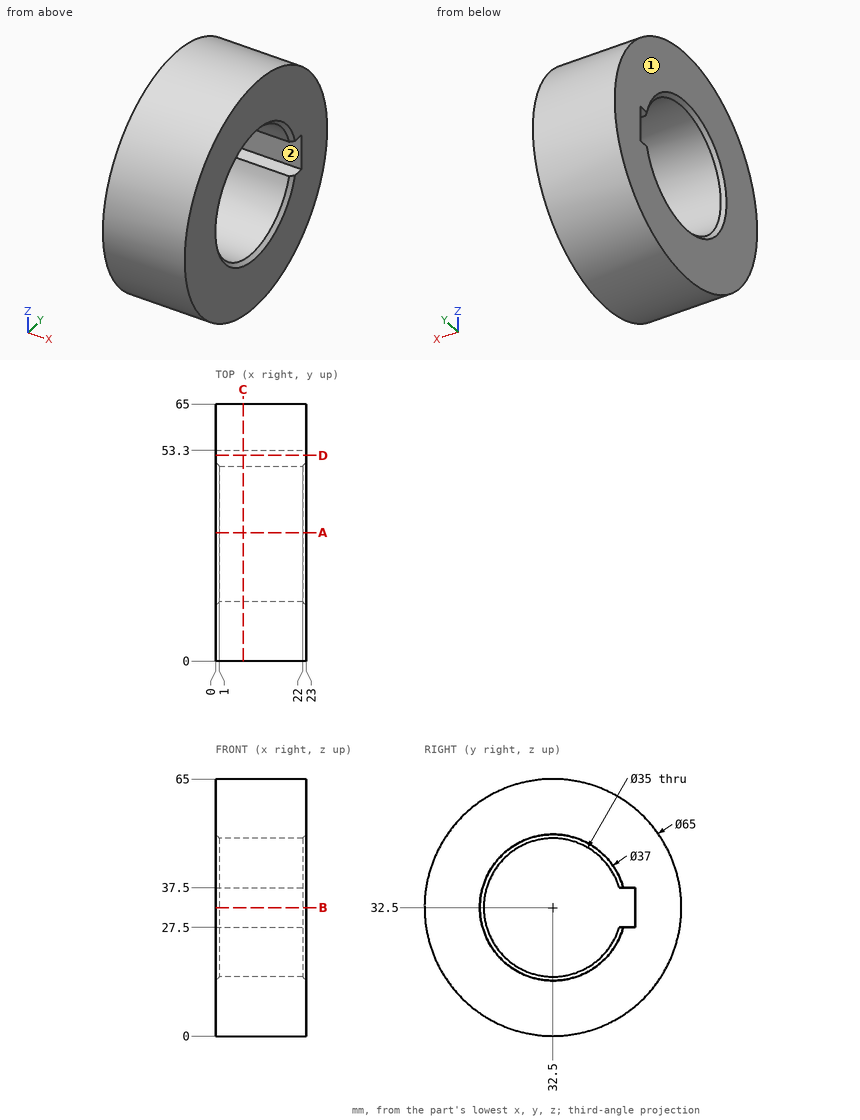
For this review, use the dimensioned drawing (mm, ordinates from the lowest corner) and the shaded views. A direction names the side the tool comes from. Round coordinates to 2 decimals unless told otherwise and drop trailing zeros. Order: outer loops, then holes, each group sorted by start corner. A loop starts at its lowest first (then second) coordinate and runs counter-clockwise, first axis right, second up. Notation, with made-up numbers: M 72.5,36.25 L 105.5,36.25 A8 cw 105.5,50.25 Z; hole C 74.5,68.5 d5. An arc over 180 degrees is marked long. Use a Markdown table: item, result.
1) Consider section D-D (y = 52). Write out the cut boundary in (x, z).
Report:
| item | result |
|---|---|
| outline | M 0,6.5 L 23,6.5 L 23,27.5 L 0,27.5 Z; M 0,37.5 L 23,37.5 L 23,58.5 L 0,58.5 Z |
2) Tool access review of the marked faces 1 and 2: name each direction out of +Z, -Z, +X, -X, +Y, -Y from which nothing blocks a thin tool from reaching the whole face with its end or side.
Report:
| item | result |
|---|---|
| face 1 | +Z, -Z, -X, +Y, -Y |
| face 2 | +X, -X |
3) Consider section C-C (x = 7). Write out the cut boundary in (y, z), then the cut area to 3 significant figures.
Report:
| item | result |
|---|---|
| outline | C 32.5,32.5 d65; hole M 49.27,27.5 L 53.3,27.5 L 53.3,37.5 L 49.27,37.5 A17.5 ccw long Z |
| area | 2,320 mm^2 |
4) Consider section B-B (z = 32.5). Write out the cut boundary in (x, y), then the cut area to 3 significant figures.
Report:
| item | result |
|---|---|
| outline | M 0,0 L 23,0 L 23,14 L 22,15 L 1,15 L 0,14 Z; M 0,53.3 L 23,53.3 L 23,65 L 0,65 Z |
| area | 613 mm^2 |
5) Consider section A-A (y = 32.5). Write out the cut boundary in (x, z).
Report:
| item | result |
|---|---|
| outline | M 0,0 L 23,0 L 23,14 L 22,15 L 1,15 L 0,14 Z; M 0,51 L 1,50 L 22,50 L 23,51 L 23,65 L 0,65 Z |
6) Wall thickness on line 1 along Y through (x, z) = (7, 32.5); line 2 along Z through (x, y) = (2.75, 50); line 3 along Y through (x, z) = (7.5, 21): over which ranges is each line inside the solid? List them lowest first. Write a range as [from, to].
Report:
| item | result |
|---|---|
| line 1 | [0, 15], [53.3, 65] |
| line 2 | [5.11, 27.5], [37.5, 59.89] |
| line 3 | [2.1, 19.31], [45.69, 62.9] |
7) Insertion check: pin 1 (6 mm diameter, centred on x = 19.5, z = 37.5, fed in from +Y); pin 2 (1.2 mm diameter, centred on x = 8, y = 52, fed in from +Z); pin 3 (1.2 mm diameter, centred on x = 9.5, y = 51, fed in from -Z); pin 4 (5 mm diameter, centred on y = 37, z = 17, fed in from +X). Each pin has a flat end and moves straight along its axis. Give the tip position at first contact, or say it passes through.
Report:
| item | result |
|---|---|
| pin 1 | y = 64.94 |
| pin 2 | z = 58.94 |
| pin 3 | z = 5.37 |
| pin 4 | x = 23 |
